Here's how the part is built. I have some questions about the finished solid (model axes, mm). A direction names the side the tool comes from. Give positions to 0.01 mm unless a question says otherwise; leave off trailing zeros. Write each loop counter-clockwise with the first axis right and the second up, starting at its lowest first coordinate (ties: lowest second). Pieces come first, ordered by that corner, then holes. Notation, with made-up numbers: (-26, -40) -> (15, -40) arc R25 ccw to (15, -1) -> close; hole circle Ø9 at (-8.75, -33). An arc over 180 degrees is marked (long way). Use CSV: the item, a comma, the result in double quotes. Start each with the question number.
(1) Which directions (+Z, -Z, +X, -X, +Y, -Y) give clear straight access to the entire face, cutting with the end or side of a thin tool? Please do faces 4 (the flat face through (0, -21, 1085)), 5 (the flat face through (-3, 22, 37)).
(2) If we mould it in two halves opening along Y, with no side actions, what happens to faces 1 (the flat face through (36, 0, 1086)), 2 (the flat face through (-40, 0, 1085)), 3 (the flat face through (0, 25, 1085))? For each: pulls with the +Y half, pulls with the -Y half, needs draft (parallel to the pull), parting line crosses it, or undercut.
(3) I need wall thicknesses on L1, parallel to X at y = -1, z = 1216; L2, parallel to Y at x = -4.5, z = 1660; L3, parallel to Y at x = 37, z = 1568. Which ranges of each line are inside material? Lowest first, please. Write a range as [from, to].
(4) Suppose I cut it at A-A on x = 10. List the corners of the cut face in (y, z) for me.
(5) Suppose I cut it at B-B on y = -11.5. List the corners of the cut face in (x, z) for me, plus the area to 3 significant figures.
(6) Suppose I cut it at C-C on z = 424.5. List the corners of the cut face in (x, y) for me, plus the area to 3 significant figures.
from build123d import *

# Parameters (mm, degrees)
BOSS_EXTRUDE1_DEPTH = 2200
SHELL1_T            = -4
CUT_EXTRUDE2_DEPTH  = 2000


with BuildPart() as part:
    # Sketch1 → Boss-Extrude1 (new body)
    with BuildSketch(Plane.XY):
        with BuildLine():
            Line((35, 25), (-35, 25))
            ThreePointArc((-35, 25), (-38.535533906, 23.535533906), (-40, 20))
            Line((-40, 20), (-40, -20))
            ThreePointArc((-40, -20), (-38.535533906, -23.535533906), (-35, -25))
            Line((-35, -25), (35, -25))
            ThreePointArc((35, -25), (38.535533906, -23.535533906), (40, -20))
            Line((40, -20), (40, 20))
            ThreePointArc((40, 20), (38.535533906, 23.535533906), (35, 25))
        make_face()
    extrude(amount=BOSS_EXTRUDE1_DEPTH)

    # Shell1
    shell1_openings = [part.faces().sort_by_distance(p)[0] for p in [
        (0, 0, 2200),
        (0, 0, 0),
    ]]
    offset(amount=SHELL1_T, openings=shell1_openings, kind=Kind.INTERSECTION)

    # Sketch3 → Cut-Extrude2 (cut)
    with BuildSketch(Plane.XZ.offset(25)):
        Polygon((-40, 2200), (40, 2120), (40, 2200), align=None)
        Polygon((40, 80), (40, 0), (-40, 0), align=None)
    extrude(amount=-CUT_EXTRUDE2_DEPTH, mode=Mode.SUBTRACT)


solid = part.part
Geometry says:
1,face 4,"+Z, -Z"
1,face 5,"-Z, +X, +Y, -Y"
2,face 1,"undercut"
2,face 2,"needs draft"
2,face 3,"pulls with the +Y half"
3,L1,"[-40, -36], [36, 40]"
3,L2,"[-25, -21], [21, 25]"
3,L3,"[-24.58, 24.58]"
4,outline,"(-25, 50) -> (-21, 50) -> (-21, 2150) -> (-25, 2150) -> close; (21, 50) -> (25, 50) -> (25, 2150) -> (21, 2150) -> close"
5,outline,"(-40, 0) -> (-36, 4) -> (-36, 2196) -> (-40, 2200) -> close; (36, 76) -> (40, 80) -> (40, 2120) -> (36, 2124) -> close"
5,area,"17,000 mm²"
6,outline,"(-40, -20) arc R5 ccw to (-35, -25) -> (35, -25) arc R5 ccw to (40, -20) -> (40, 20) arc R5 ccw to (35, 25) -> (-35, 25) arc R5 ccw to (-40, 20) -> close; hole (-36, -20) arc R1 ccw to (-35, -21) -> (35, -21) arc R1 ccw to (36, -20) -> (36, 20) arc R1 ccw to (35, 21) -> (-35, 21) arc R1 ccw to (-36, 20) -> close"
6,area,"955 mm²"
